```python
from build123d import *

# Parameters (mm, degrees)
SKETCH1_W           = 130
SKETCH1_H           = 460
BOSS_EXTRUDE1_DEPTH = 10
CUT_EXTRUDE1_DEPTH  = 240.843699104


with BuildPart() as part:
    # Sketch1 → Boss-Extrude1 (new, symmetric)
    with BuildSketch(Plane.XY):
        Rectangle(SKETCH1_W, SKETCH1_H)
    extrude(amount=BOSS_EXTRUDE1_DEPTH, both=True)

    # Sketch2 → Cut-Extrude1 (cut, through all)
    with BuildSketch(Plane.XY.offset(10)):
        Polygon((-65, 180), (35, -230), (-65, -230), align=None)
    extrude(amount=-CUT_EXTRUDE1_DEPTH, mode=Mode.SUBTRACT)


solid = part.part
```
Model file for the job. Use its own axes, mm. Round coordinates to 2 decimals unless told otherwise and drop trailing zeros. Write each loop counter-clockwise with the first axis right and the second up, starting at its lowest first coordinate (ties: lowest second). Pieces come first, ordered by that corner, then holes. Notation, with made-up numbers: (-23.75, 53.25) - (23.25, 53.25) arc R13 cw to (23.25, 61.25) - close; hole circle Ø3 at (-27.75, -19.5). An arc over 180 degrees is marked (long way). One line per item, written item: value.
(1) Two-plate mould, pull along X, no slides. Class faces 1 (the flat face through (50, -230, 0)), 2 (the flat face through (-65, 205, 0)), 3 (the flat face through (65, -3, 0)): pulls with the +X half, pulls with the -X half, needs draft (parallel to the pull), parting line crosses it, or undercut.
Values follow:
face 1: needs draft
face 2: pulls with the -X half
face 3: pulls with the +X half
(2) Cut at A-A, the plane z = -1.5. Give the cut face in (x, y), plus the area to 3 significant figures.
Values follow:
outline: (-65, 180) - (35, -230) - (65, -230) - (65, 230) - (-65, 230) - close
area: 39,300 mm²
(3) Drop flat-ended pins along their axis: P1, Ø4, axis at y = -157, z = 0, coming from the -X side; P2, Ø4, axis at y = 23.5, z = 0, coming from the -X side. Give the stop position or say it passes through.
Values follow:
P1: stops at x = 16.71
P2: stops at x = -27.32
(4) Cut at C-C, the plane y = -153.5. Give the cut face in (x, z), plus the area to 3 significant figures.
Values follow:
outline: (16.34, -10) - (65, -10) - (65, 10) - (16.34, 10) - close
area: 973 mm²
(5) Cut at B-B, the plane x = -55. Give the cut face in (y, z).
Values follow:
outline: (139, -10) - (230, -10) - (230, 10) - (139, 10) - close
(6) Wall check: probe 1 along X at (y, z) = (-49, -2.5); probe 2 along X at (y, z) = (40, 2). Give the ranges that are in metal, low to high.
Values follow:
probe 1: x = -9.15 to 65
probe 2: x = -30.85 to 65
